Could you check a few things on this drawing? It's one solid part, dimensions in mm from its lowest x, y, z. A direction names the side the tool comes from. Give positions to 0.01 mm unless a question says otherwise; leave off trailing zeros. Write each loop counter-clockwise with the first axis right and the second up, starting at its lowest first coordinate (ties: lowest second). Pieces come first, ordered by that corner, then holes. Notation, with made-up numbers: M 35,-11 L 61,-11 A25 ccw 61,5 Z; hole C -26.75,-12 d9. An arc over 180 degrees is marked long. Write each question's results on one line, items separated by ' | '.
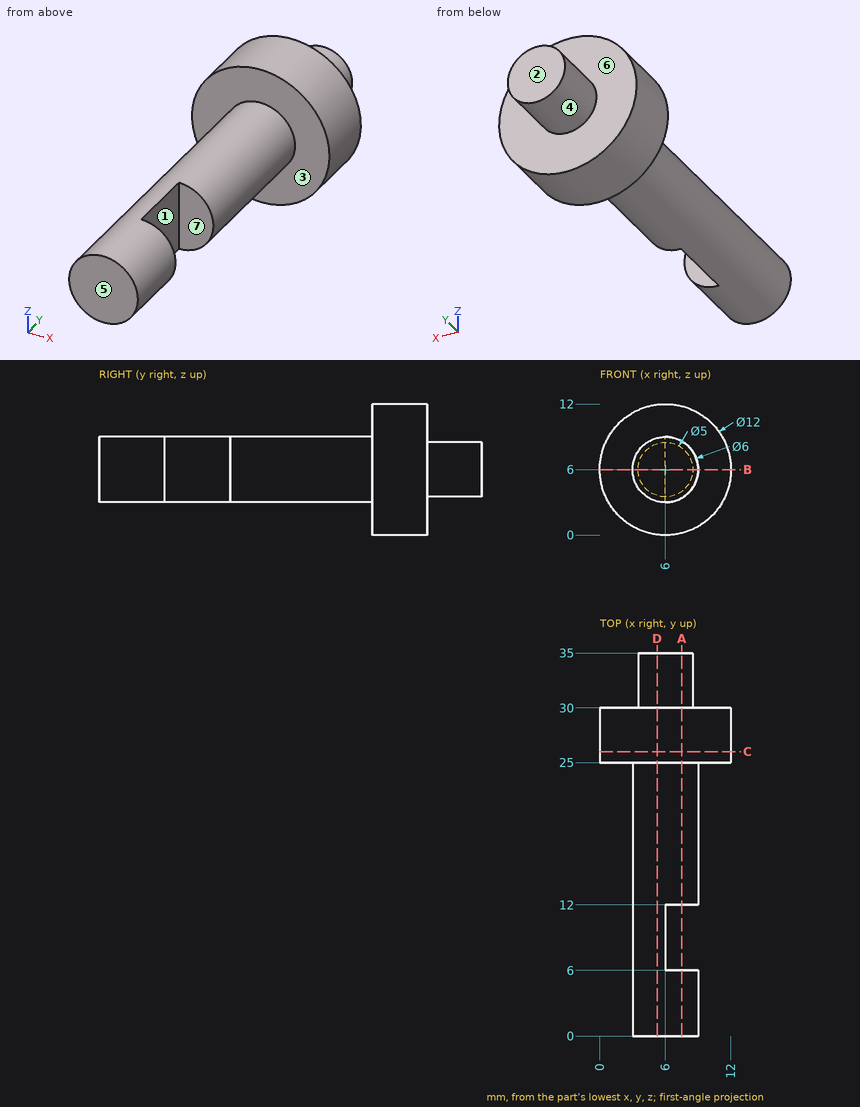
Item 1: I want a section at A-A, the plane x = 7.5. Please give me the cut outline in (y, z).
Geometry says:
outline: M 0,3.4 L 6,3.4 L 6,8.6 L 0,8.6 Z; M 12,3.4 L 25,3.4 L 25,0.19 L 30,0.19 L 30,4 L 35,4 L 35,8 L 30,8 L 30,11.81 L 25,11.81 L 25,8.6 L 12,8.6 Z
Item 2: Thinking about a two-plate mould opening in Y: for the marked faces 5, 6 and 7, which applies, +Y half, -Y half, draft (parallel to the pull), parting line (faces both ways), or undercut?
Geometry says:
face 5: -Y half | face 6: +Y half | face 7: undercut
Item 3: I want a section at B-B, the plane z = 6. Please give me the cut outline in (x, y).
Geometry says:
outline: M 0,25 L 3,25 L 3,0 L 9,0 L 9,6 L 6,6 L 6,12 L 9,12 L 9,25 L 12,25 L 12,30 L 8.5,30 L 8.5,35 L 3.5,35 L 3.5,30 L 0,30 Z
Item 4: I'm going to push flat-ended pins straight in: pin 1 (1 mm diameter, centred on y = 4.5, z = 4.5, fed in from -X); pin 2 (1 mm diameter, centred on x = 6, y = 19, fed in from +Z); pin 3 (2 mm diameter, centred on x = 9.5, z = 3.5, fed in from -Y). Where does each tip first touch, or does it pass through?
Geometry says:
pin 1: stops at x = 3.17 | pin 2: stops at z = 9 | pin 3: stops at y = 25
Item 5: I want a section at C-C, the plane y = 26. Please give me the cut outline in (x, z).
Geometry says:
outline: C 6,6 d12
Item 6: For the marked faces 1, 2, 3 and 4, which set-ups out of +Z, -Z, +X, -X, +Y, -Y let a thin tool reach every point of the face, with its end or its side?
Geometry says:
face 1: +Z, -Z, +X | face 2: +Z, -Z, +X, -X, +Y | face 3: -Y | face 4: +Y
Item 7: I want a section at D-D, the plane x = 5.25. Please give me the cut outline in (y, z).
Geometry says:
outline: M 0,3.1 L 25,3.1 L 25,0.05 L 30,0.05 L 30,3.62 L 35,3.62 L 35,8.38 L 30,8.38 L 30,11.95 L 25,11.95 L 25,8.9 L 0,8.9 Z
Item 8: If I drill on line 1 (Y direction, x = 6.5, z = 8); line 2 (Y direction, x = 9.75, z = 2.5); line 3 (Y direction, x = 3.5, z = 6.75), over which ranges is the centre line in solid material (lowest first)? Write a range as from..to.
Geometry says:
line 1: y = 0..6, 12..35 | line 2: y = 25..30 | line 3: y = 0..30
